Part print with two shaded views. Sizes in mm from the minimum x, y, z corner. Round coordinates to 2 decimals unless told otherwise and drop trailing zeros. Order: outer loops, then holes, each group sorted by start corner. A loop starts at its lowest first (then second) coordinate and runs counter-clockwise, first axis right, second up. Notation, with made-up numbers: M 15,18.5 L 46,18.5 A19 ccw 46,48.5 Z; hole C 23.5,19.25 d5. An arc over 180 degrees is marked long. Put each result on its own line as item: value.
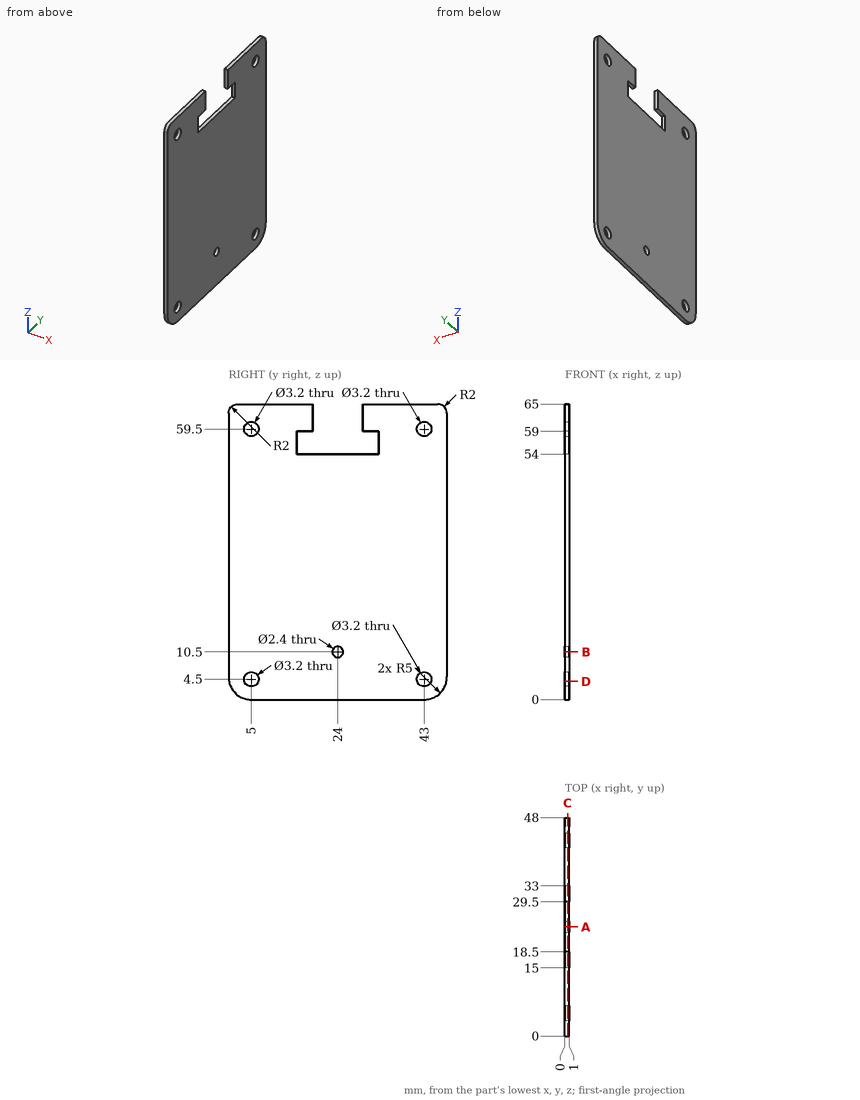
Item 1: Band-saw the part on C-C on x = 0.6. Give the cut face in (y, z), and give its area (3 significant figures).
Answers below:
outline: M 0,5 A5 ccw 5,0 L 43,0 A5 ccw 48,5 L 48,63 A2 ccw 46,65 L 29.5,65 L 29.5,59 L 33,59 L 33,54 L 15,54 L 15,59 L 18.5,59 L 18.5,65 L 2,65 A2 ccw 0,63 Z; hole C 5,4.5 d3.2; hole C 5,59.5 d3.2; hole C 24,10.5 d2.4; hole C 43,4.5 d3.2; hole C 43,59.5 d3.2
area: 2,910 mm²
Item 2: Band-saw the part on A-A on y = 24. Give the cut face in (x, z), and give its area (3 significant figures).
Answers below:
outline: M 0,0 L 1,0 L 1,9.3 L 0,9.3 Z; M 0,11.7 L 1,11.7 L 1,54 L 0,54 Z
area: 51.6 mm²
Item 3: Pin check, flat tip, straight feed: P1, Ø2.5, axis at y = 5, z = 4.5, coming from the +X side. Stop position of the tip, or through.
Answers below:
P1: through
Item 4: Probe line 1 along Y through (x, z) = (0.75, 59.5); line 2 along Y through (x, z) = (0.25, 4.5); line 3 along Z through (x, y) = (0.5, 25.5). List the from-to ranges inside material, lowest first. Write a range as [from, to].
Answers below:
line 1: [0, 3.4], [6.6, 18.5], [29.5, 41.4], [44.6, 48]
line 2: [0.03, 3.4], [6.6, 41.4], [44.6, 47.97]
line 3: [0, 54]
Item 5: Band-saw the part on B-B on z = 10.5. Give the cut face in (x, y).
Answers below:
outline: M 0,0 L 1,0 L 1,22.8 L 0,22.8 Z; M 0,25.2 L 1,25.2 L 1,48 L 0,48 Z
Item 6: Band-saw the part on D-D on z = 4. Give the cut face in (x, y).
Answers below:
outline: M 0,0.1 L 1,0.1 L 1,3.48 L 0,3.48 Z; M 0,6.52 L 1,6.52 L 1,41.48 L 0,41.48 Z; M 0,44.52 L 1,44.52 L 1,47.9 L 0,47.9 Z
